Part print with two shaded views. Sizes in mm from the minimum x, y, z corner. A direction names the side the tool comes from. Coordinates: 2 decimals unless noted, no trailing zeros. Loops run counter-clockwise (first coordinate to the right, second up) from the corner with the lowest first, then second, coordinate; pieces in that order, holes last. Notation, with made-up numbers: (62, 71) -> (110, 71) arc R22 cw to (110, 101) -> close; hole circle Ø8 at (-4, 12.5). An arc over 180 degrees is marked (long way). Use one line per item in the form item = value.
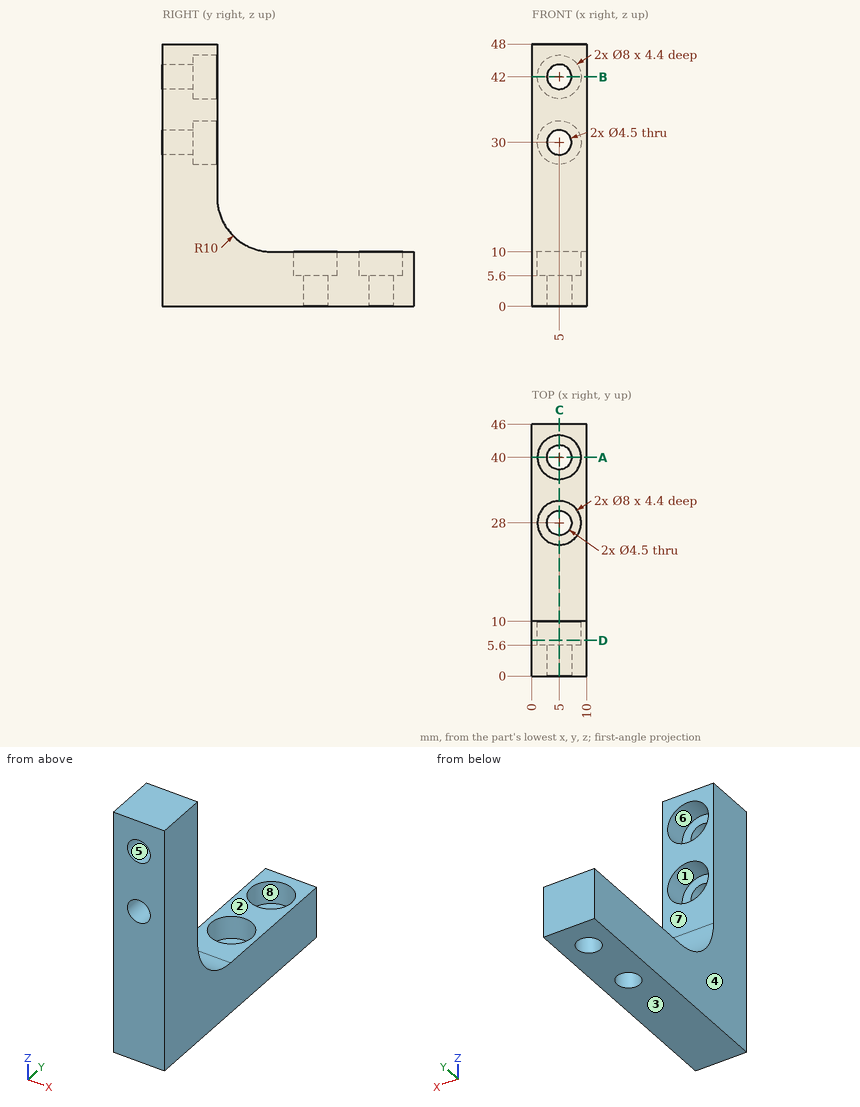
Q1. Wall check: line 1 along Y through (x, z) = (5, 3); line 2 along Z through (x, y) = (4.75, 9); line 3 along X through (y, z) = (7.8, 30). Give the ranges that are in metal, low to high.
Result:
line_1 = 0 to 25.75, 30.25 to 37.75, 42.25 to 46
line_2 = 0 to 26.01, 33.99 to 38.01, 45.99 to 48
line_3 = 0 to 1, 9 to 10
Q2. Pin check, flat tips, straight feed: pin 1 Ø5 at (x, y) = (5, 40) entering from +Z; pin 2 Ø5 at (x, y) = (4.5, 29.5) entering from +Z; pin 3 Ø4 at (x, z) = (4.5, 41.5) entering from +Y. Stop position of each tip, or through.
Result:
pin_1 = 5.6
pin_2 = 10
pin_3 = 5.6
Q3. Band-saw the part on A-A, the plane y = 40. Write the cut outline in (x, z).
Result:
outline = (0, 0) -> (2.75, 0) -> (2.75, 5.6) -> (1, 5.6) -> (1, 10) -> (0, 10) -> close; (7.25, 0) -> (10, 0) -> (10, 10) -> (9, 10) -> (9, 5.6) -> (7.25, 5.6) -> close
Q4. Which spindle directions (+Z, -Z, +X, -X, +Y, -Y) get a long thin tool onto all of the face, cutting with end or side? Do the marked faces 4, 5, 6, 7 and 8. Say none if no direction does.
Result:
face_4 = +Z, -Z, -X, +Y, -Y
face_5 = +Y, -Y
face_6 = +Y
face_7 = +Z, +X, -X, +Y
face_8 = +Z
Q5. Mould opens along Z. For the marked faces 1, 2 and 3 say: released by +Z, released by -Z, zero draft, split by the parting line, or undercut.
Result:
face_1 = undercut
face_2 = released by +Z
face_3 = released by -Z
Q6. Band-saw the part on D-D, the plane y = 6.5. Write the cut outline in (x, z).
Result:
outline = (0, 0) -> (10, 0) -> (10, 48) -> (0, 48) -> close; hole circle Ø8 at (5, 30); hole circle Ø8 at (5, 42)
Q7. Band-saw the part on C-C, the plane x = 5. State how many separate pieces and enclosed holes the cut face has, and give its area (3 significant figures).
Result:
separate_pieces = 5
enclosed_holes = 0
area = 620 mm2
